Can you work these out from the model? Positions are in its coordinate system, mm. A direction names the side the tool comes from. Round coordinates to 2 decimals unless told otherwise and drop trailing zeros. Write each loop counter-clockwise with the first axis right and the second up, starting at its lowest first coordinate (ties: lowest second). Pieces come first, ordered by that corner, then holes. Notation, with made-up numbers: (-23.5, 87) - (26.5, 87) arc R30 cw to (26.5, 119) - close; hole circle Ø6 at (34, 14.25). An arc over 180 degrees is marked (long way). One line per item, written item: value. Start each with the question number.
(1) I want a section at B-B on x = 2.5. List the corners of the cut face in (y, z) for me.
(2) If I drill on L1, parallel to Y at x = 14.5, z = 0; L2, parallel to X at y = 1.75, z = -0.25; L3, parallel to Y at x = 10.5, z = -1, over which ranges is the centre line in solid material (lowest first)? Write a range as from..to.
(3) On a 3-axis mill with a long thin cutter (end or side, diameter ignored), from which of +Z, -Z, +X, -X, +Y, -Y can I reach the whole of each face in a straight line? I mean faces 1 (the face through (0.805, -0.937, 2.976)), 2 (the face through (1.6, 0, 2)). Say none if no direction works.
(4) I'm going to push flat-ended pins straight in: pin 1 Ø1.5 at (x, z) = (13, 2) entering from +Y; pin 2 Ø1 at (x, z) = (13.5, 0.5) entering from +Y. Where does each tip first touch, or does it pass through?
(5) I want a section at A-A on z = 0. List the corners of the cut face in (x, y) for me.
from build123d import *


with BuildPart() as part:
    # Dimensioned Sketch → Revolve3 (revolve)
    with BuildSketch(Plane.XY, mode=Mode.PRIVATE) as revolve3_sk:
        with BuildLine():
            Line((0, 0), (0, 2.6752))
            ThreePointArc((0, 2.6752), (0.130278904, 2.989721096), (0.4448, 3.12))
            Line((0.4448, 3.12), (1.1552, 3.12))
            ThreePointArc((1.1552, 3.12), (1.469721096, 2.989721096), (1.6, 2.6752))
            Line((1.6, 2.6752), (1.6, 1.6))
            ThreePointArc((1.6, 1.6), (1.629289322, 1.529289322), (1.7, 1.5))
            Line((1.7, 1.5), (15.6, 1.5))
            Line((15.6, 1.5), (15.6, 0))
            Line((15.6, 0), (0, 0))
        make_face()
    revolve(revolve3_sk.sketch.rotate(Axis((0, 0, 0), (1, 0, 0)), 90), axis=Axis((0, 0, 0), (1, 0, 0)))


solid = part.part
Established:
1. outline: circle Ø3 at (0, 0)
2. L1: -1.5..1.5
2. L2: 0..1.6
2. L3: -1.12..1.12
3. face 1: +X, -X
3. face 2: +X
4. pin 1: y = 0.83
4. pin 2: y = 1.5
5. outline: (0, -2.68) arc R0.44 ccw to (0.44, -3.12) - (1.16, -3.12) arc R0.44 ccw to (1.6, -2.68) - (1.6, -1.6) arc R0.1 cw to (1.7, -1.5) - (15.6, -1.5) - (15.6, 1.5) - (1.7, 1.5) arc R0.1 cw to (1.6, 1.6) - (1.6, 2.68) arc R0.44 ccw to (1.16, 3.12) - (0.44, 3.12) arc R0.44 ccw to (0, 2.68) - close
